Can you work these out from the model? Positions are in its coordinate system, mm. Round coordinates to 2 decimals unless told otherwise and drop trailing zeros. Order: outer loops, then holes, each group sorted by start corner. A loop starts at its lowest first (then second) coordinate and runs counter-clockwise, first axis right, second up. Notation, with made-up numbers: M 46,44 L 85,44 A22 cw 85,69 Z; hole C 19.25,51.25 d8. An arc over 180 degrees is marked long. Answer as a JSON object with one key per item and string values. Group by question number.
from build123d import *

# Parameters (mm, degrees)
SKETCH1_W           = 240
SKETCH1_H           = 140
SKETCH1_R           = 25.5
BOSS_EXTRUDE1_DEPTH = 25


with BuildPart() as part:
    # Sketch1 → Boss-Extrude1 (new body)
    with BuildSketch(Plane.XY):
        with Locations((120, 70)):
            Rectangle(SKETCH1_W, SKETCH1_H)
        with Locations((120, 59)):
            Circle(SKETCH1_R, mode=Mode.SUBTRACT)
    extrude(amount=BOSS_EXTRUDE1_DEPTH)


solid = part.part
Item 1: Suppose I cut it at A-A, the plane x = 120. Write out the boundary of the cut face in (y, z).
Item 2: If we mould it in two halves opening along X, with no side actions, what happens to faces 1 (the face through (240, 69, 12)), 2 (the face through (99.764, 43.484, 12.325)), 3 (the face through (118, 87, 25))? For each: +X half, -X half, draft (parallel to the pull), parting line (faces both ways), or undercut.
Item 3: Suppose I cut it at B-B, the plane y = 59. Write out the boundary of the cut face in (x, z), and give its area (4 significant figures).
Item 4: Suppose I cut it at C-C, the plane z = 4. Write out the boundary of the cut face in (x, y).
Item 5: I need wall thicknesses on line 1 (Y direction, x = 120, z = 11.75); line 2 (X direction, y = 82, z = 14.75); line 3 (X direction, y = 41, z = 14.75). Which ranges of each line are inside material? Lowest first, please.
Item 6: I'm going to push a flat-ended pin straight in: pin 1 Ø4 at (x, y) = (58, 21) entering from -Z. Where does the tip first touch, or does it pass through?
Computed:
{
 "1": {"outline": "M 0,0 L 33.5,0 L 33.5,25 L 0,25 Z; M 84.5,0 L 140,0 L 140,25 L 84.5,25 Z"},
 "2": {"face 1": "+X half", "face 2": "undercut", "face 3": "draft"},
 "3": {"outline": "M 0,0 L 94.5,0 L 94.5,25 L 0,25 Z; M 145.5,0 L 240,0 L 240,25 L 145.5,25 Z", "area": "4,725 mm^2"},
 "4": {"outline": "M 0,0 L 240,0 L 240,140 L 0,140 Z; hole C 120,59 d51"},
 "5": {"line 1": "y = 0 to 33.5, 84.5 to 140", "line 2": "x = 0 to 108.99, 131.01 to 240", "line 3": "x = 0 to 101.94, 138.06 to 240"},
 "6": {"pin 1": "stops at z = 0"}
}
